Check sheet for the modelled part. Datum: model origin and axes. Units: mm. A direction names the side the tool comes from. Round coordinates to 2 decimals unless told otherwise and drop trailing zeros. Loops run counter-clockwise (first coordinate to the right, second up) from the corner with the lowest first, then second, coordinate; pieces in that order, holes last. Notation, with made-up numbers: (80.5, -8) -> (102.5, -8) arc R22 ccw to (102.5, 28) -> close; hole circle Ø11 at (40.5, -39). An arc over 180 degrees is marked (long way). One line per item, written item: value. Start each with the question number.
1. Cross-section at C-C on y = -18.84. Record the cut outline in (x, z), then the cut area to 3 significant figures.
2. Cross-section at A-A on y = -26. Record the cut outline in (x, z), then the cut area to 3 significant figures.
3. Release check for a two-part mould opening along Z. For faces 1 (the face through (19, -22, -5.5)), 2 (the face through (35.067, -6.375, 9.049)), 3 (the face through (-37, -27, 4.5)) record: +Z half, -Z half, draft (parallel to the pull), parting line (faces both ways), or undercut.
4. Set-up check for faces 4 (the face through (-32, -40.539, -4)), 5 (the face through (11.39, -31.42, 0.08)), 6 (the face through (-20.468, -24, 9)): record each of +Z, -Z, +X, -X, +Y, -Y from which the full face is reachable in a straight line by a thin tool's end or side.
5. Go/stop test with flat-tipped pins: pin 1 (3 mm diameter, centred on y = -48, z = 2.5, fed in from +X); pin 2 (3 mm diameter, centred on x = -34.5, y = -25.5, fed in from +Z); pin 3 (1.5 mm diameter, centred on x = -16.5, z = -3.5, fed in from -Y); pin 4 (2.5 mm diameter, centred on y = -19.5, z = 8.5, fed in from -X). Record where each tip stops, or that it passes through.
6. Cross-section at B-B on z = 9. Record the cut outline in (x, y), then the cut area to 3 significant figures.
7. Cross-section at D-D on x = 8. Record the cut outline in (y, z), then the cut area to 3 significant figures.
8. Material ranges on L1, parallel to X at y = -18.84, z = 10.5; L2, parallel to Z at x = 33, y = -21; L3, parallel to X at y = -18.84, z = -8, recorded low to high.
from build123d import *

# Parameters (mm, degrees)
BRACKET_PROFILE_SKETCH_R   = 5
BRACKET_PROFILE_SKETCH_R_2 = 7
BRACKET_BODY_25MM_DEPTH    = 12.5
FORK_SLOT_SKETCH_W         = 27
FORK_SLOT_SKETCH_H         = 8
FORK_SLOT_8X27_DEPTH       = 63
RELIEF_CIRCLE_SKETCH_76_R  = 38
FRONT_RELIEF_CUT_76_DEPTH  = 5.5


with BuildPart() as part:
    # Bracket Profile Sketch → Bracket Body 25mm (new, symmetric)
    with BuildSketch(Plane.XY):
        with BuildLine():
            Line((-1.467633793, -60.539351202), (11.532366207, -60.539351202))
            Line((11.532366207, -60.539351202), (37.532366207, -28.84))
            Line((37.532366207, -28.84), (37.532366207, -8.84))
            Line((37.532366207, -8.84), (32.532366207, -3.84))
            Line((32.532366207, -3.84), (15.532366207, -3.84))
            ThreePointArc((15.532366207, -3.84), (6.522255442, -14.610276655), (-7.511545005, -14.127161486))
            Line((-7.511545005, -14.127161486), (-19.901414154, -7.539351202))
            Line((-19.901414154, -7.539351202), (-42.467633793, -7.539351202))
            Line((-42.467633793, -7.539351202), (-47.467633793, -12.539351202))
            Line((-47.467633793, -12.539351202), (-47.467633793, -35.539351202))
            Line((-47.467633793, -35.539351202), (-42.467633793, -40.539351202))
            Line((-42.467633793, -40.539351202), (-20.467867574, -40.539351202))
            ThreePointArc((-20.467867574, -40.539351202), (-14.992702243, -42.171402553), (-11.304687106, -46.534838282))
            ThreePointArc((-11.304687106, -46.534838282), (-7.089928905, -54.031435949), (-1.467633793, -60.539351202))
        make_face()
        with Locations((25.532366207, -18.84)):
            Circle(BRACKET_PROFILE_SKETCH_R, mode=Mode.SUBTRACT)
        with Locations((-31.467633793, -21.539351202)):
            Circle(BRACKET_PROFILE_SKETCH_R_2, mode=Mode.SUBTRACT)
    extrude(amount=BRACKET_BODY_25MM_DEPTH, both=True)

    # Fork Slot Sketch → Fork Slot 8x27 (cut)
    with BuildSketch(Plane(origin=(0, 0, 0), x_dir=(1, 0, 0), z_dir=(0, 1, 0))):
        with Locations((-33.967633793, -8.5)):
            Rectangle(FORK_SLOT_SKETCH_W, FORK_SLOT_SKETCH_H)
    extrude(amount=-FORK_SLOT_8X27_DEPTH, mode=Mode.SUBTRACT)

    # Relief Circle Sketch Ø76 → Front Relief Cut Ø76 (cut, symmetric)
    with BuildSketch(Plane.XY):
        with Locations((37.532366207, -3.84)):
            Circle(RELIEF_CIRCLE_SKETCH_76_R)
    extrude(amount=FRONT_RELIEF_CUT_76_DEPTH, both=True, mode=Mode.SUBTRACT)


solid = part.part
Taken from the geometry:
1. outline: (-47.47, -12.5) -> (-37.93, -12.5) -> (-37.93, 4.5) -> (-47.47, 4.5) -> close; (-25.01, -12.5) -> (20.53, -12.5) -> (20.53, -5.5) -> (2.62, -5.5) -> (2.62, 5.5) -> (20.53, 5.5) -> (20.53, 12.5) -> (-20.47, 12.5) -> (-20.47, 4.5) -> (-25.01, 4.5) -> close; (30.53, -12.5) -> (37.53, -12.5) -> (37.53, -5.5) -> (30.53, -5.5) -> close; (30.53, 5.5) -> (37.53, 5.5) -> (37.53, 12.5) -> (30.53, 12.5) -> close
1. area: 1,170 mm2
2. outline: (-47.47, -12.5) -> (-36.86, -12.5) -> (-36.86, 4.5) -> (-47.47, 4.5) -> close; (-26.07, -12.5) -> (37.53, -12.5) -> (37.53, -5.5) -> (6.66, -5.5) -> (6.66, 5.5) -> (37.53, 5.5) -> (37.53, 12.5) -> (-20.47, 12.5) -> (-20.47, 4.5) -> (-26.07, 4.5) -> close
2. area: 1,390 mm2
3. face 1: undercut
3. face 2: draft
3. face 3: +Z half
4. face 4: +Z, -Z, -X, -Y
4. face 5: +X, +Y
4. face 6: +Z, -X, +Y, -Y
5. pin 1: stops at x = 23.05
5. pin 2: passes through
5. pin 3: stops at y = -41.72
5. pin 4: stops at x = -20.47
6. outline: (-20.47, -40.54) arc R10 cw to (-11.3, -46.53) arc R43 ccw to (-1.47, -60.54) -> (11.53, -60.54) -> (37.53, -28.84) -> (37.53, -8.84) -> (32.53, -3.84) -> (15.53, -3.84) arc R16 cw to (-7.51, -14.13) -> (-19.9, -7.54) -> (-20.47, -7.54) -> close; hole circle Ø10 at (25.53, -18.84)
6. area: 2,240 mm2
7. outline: (-60.54, -12.5) -> (-13.86, -12.5) -> (-13.86, -5.5) -> (-27.75, -5.5) -> (-27.75, 5.5) -> (-13.86, 5.5) -> (-13.86, 12.5) -> (-60.54, 12.5) -> close
7. area: 1,010 mm2
8. L1: x = -20.47 to 20.53, 30.53 to 37.53
8. L2: z = -12.5 to -5.5, 5.5 to 12.5
8. L3: x = -47.47 to -37.93, -25.01 to 20.53, 30.53 to 37.53
